```python
from build123d import *

# Parameters (mm, degrees)
TRIANGULAR_BASE_PLATE_DEPTH   = 10
TUBE_SUPPORT_BLOCK_PROFILE_W  = 16
TUBE_SUPPORT_BLOCK_PROFILE_H  = 10
TUBE_SUPPORT_BLOCK_DEPTH      = 55
SUPPORT_WEB_PROFILE_W         = 16
SUPPORT_WEB_PROFILE_H         = 6
SUPPORT_WEB_DEPTH             = 55
TUBE_PROFILE_32_R             = 16
ROUND_TUBE_32_DEPTH           = 55
TUBE_START                    = 30
TUBE_EXTENSION_PROFILE_32_R   = 16
TUBE_EXTENSION_32_DEPTH       = 30
TUBE_BORE_PROFILE_21_R        = 10.5
TUBE_BORE_21_DEPTH            = 85
MOUNTING_HOLES_PROFILE_3X_8_R = 4
MOUNTING_HOLES_3X_8_DEPTH     = 85


with BuildPart() as part:
    # Base Plate Profile → Triangular Base Plate (new body)
    with BuildSketch(Plane.XY):
        with BuildLine():
            Line((-50.21997456, -52.0500159), (-12.71997456, 7.9499841))
            ThreePointArc((-12.71997456, 7.9499841), (0, 15), (12.71997456, 7.9499841))
            Line((12.71997456, 7.9499841), (50.21997456, -52.0500159))
            ThreePointArc((50.21997456, -52.0500159), (50.619637219, -67.271527986), (37.5, -75))
            Line((37.5, -75), (-37.5, -75))
            ThreePointArc((-37.5, -75), (-50.619637219, -67.271527986), (-50.21997456, -52.0500159))
        make_face()
    extrude(amount=TRIANGULAR_BASE_PLATE_DEPTH)

    # Tube Support Block Profile → Tube Support Block (add)
    with BuildSketch(Plane.XZ.offset(75)):
        with Locations((-8, 15)):
            Rectangle(TUBE_SUPPORT_BLOCK_PROFILE_W, TUBE_SUPPORT_BLOCK_PROFILE_H)
        with Locations((8, 15)):
            Rectangle(TUBE_SUPPORT_BLOCK_PROFILE_W, TUBE_SUPPORT_BLOCK_PROFILE_H)
    extrude(amount=-TUBE_SUPPORT_BLOCK_DEPTH)

    # Support Web Profile → Support Web (add)
    with BuildSketch(Plane.XZ.offset(75)):
        with Locations((-8, 23)):
            Rectangle(SUPPORT_WEB_PROFILE_W, SUPPORT_WEB_PROFILE_H)
        with Locations((8, 23)):
            Rectangle(SUPPORT_WEB_PROFILE_W, SUPPORT_WEB_PROFILE_H)
    extrude(amount=-SUPPORT_WEB_DEPTH)

    # Tube Profile Ø32 → Round Tube Ø32 (add)
    with BuildSketch(Plane.XZ.offset(75)):
        with Locations((0, 26)):
            Circle(TUBE_PROFILE_32_R)
    extrude(amount=-ROUND_TUBE_32_DEPTH)

    # Tube Extension Profile Ø32 → Tube Extension Ø32 (add)
    with BuildSketch(Plane.XZ.offset(75).offset(TUBE_START)):
        with Locations(Location((0, 26, 0), (0, 0, 270))):
            Circle(TUBE_EXTENSION_PROFILE_32_R)
    extrude(amount=-TUBE_EXTENSION_32_DEPTH)

    # Tube Bore Profile Ø21 → Tube Bore Ø21 (cut)
    with BuildSketch(Plane.XZ.offset(105)):
        with Locations(Location((0, 26, 0), (0, 0, 270))):
            Circle(TUBE_BORE_PROFILE_21_R)
    extrude(amount=-TUBE_BORE_21_DEPTH, mode=Mode.SUBTRACT)

    # Mounting Holes Profile 3xØ8 → Mounting Holes 3xØ8 (cut)
    with BuildSketch(Plane.XY.offset(10)):
        Circle(MOUNTING_HOLES_PROFILE_3X_8_R)
        with Locations((-37.5, -60)):
            Circle(MOUNTING_HOLES_PROFILE_3X_8_R)
        with Locations((37.5, -60)):
            Circle(MOUNTING_HOLES_PROFILE_3X_8_R)
    extrude(amount=-MOUNTING_HOLES_3X_8_DEPTH, mode=Mode.SUBTRACT)


solid = part.part
```
Work out the finished part from the listing and answer in its coordinate system (mm). A direction names the side the tool comes from. Coordinates: 2 decimals unless noted, no trailing zeros. Loops run counter-clockwise (first coordinate to the right, second up) from the corner with the lowest first, then second, coordinate; pieces in that order, holes last.
1) Flat-ended cylindrical pins translate along their axes: pin 1 (1.5 mm diameter, centred on x = 14, y = -49, fed in from -Z); pin 2 (5 mm diameter, centred on y = -42.5, z = 19.5, fed in from -X); pin 3 (1 mm diameter, centred on y = -80.5, z = 27.5, fed in from +X); pin 4 (1.5 mm diameter, centred on x = -23, y = -39, fed in from +Z). Find the tip coordinate at first contact, or state that the pin passes through.
Results:
pin 1: stops at z = 0
pin 2: stops at x = -16
pin 3: stops at x = 15.97
pin 4: stops at z = 10
2) Section D-D (y = -47.5) is taken. Give the vertices of the cut face in (x, z), plus the area to 3 significant figures.
Results:
outline: (-47.38, 0) - (47.38, 0) - (47.38, 10) - (16, 10) - (16, 26) arc R16 ccw to (-16, 26) - (-16, 10) - (-47.38, 10) - close; hole circle Ø21 at (0, 26)
area: 1,520 mm2
3) Consider probe 1 along Z at (x, y) = (0.5, -99); probe 2 along X at (y, z) = (-79, 26); probe 3 along Z at (x, y) = (-25, -43). Determine where each line is inside the solid, lowest interval first.
Results:
probe 1: z = 10.01 to 15.51, 36.49 to 41.99
probe 2: x = -16 to -10.5, 10.5 to 16
probe 3: z = 0 to 10
4) Section B-B (x = 0) is taken. Give the vertices of the cut face in (y, z), plus the area to 4 significant figures.
Results:
outline: (-105, 10) - (-75, 10) - (-75, 0) - (-4, 0) - (-4, 10) - (-20, 10) - (-20, 15.5) - (-105, 15.5) - close; (-105, 36.5) - (-20, 36.5) - (-20, 42) - (-105, 42) - close; (4, 0) - (15, 0) - (15, 10) - (4, 10) - close
area: 1,755 mm2
5) Section C-C (z = 17.5) is taken. Give the vertices of the cut face in (x, y), plus the area to 3 significant figures.
Results:
outline: (-16, -75) - (-13.56, -75) - (-13.56, -105) - (-6.16, -105) - (-6.16, -20) - (-16, -20) - close; (6.16, -105) - (13.56, -105) - (13.56, -75) - (16, -75) - (16, -20) - (6.16, -20) - close
area: 1,530 mm2
6) For faces 4 (the flat face through (3.3, -20, 15.6)), 5 (the flat face through (-16, -48, 18)), 6 (the cylindrical face through (0, 15, 5)), 7 (the flat face through (16, -48, 18)), 8 (the cylindrical face through (0.703, -72.539, 41.985)), determine the directions among +Z, -Z, +X, -X, +Y, -Y from which every point of the face is accessible in a straight line to the end or side of a thin tool.
Results:
face 4: +Z, +X, -X, +Y
face 5: +Z, -X, +Y, -Y
face 6: +Z, -Z, +Y
face 7: +Z, +X, +Y, -Y
face 8: -Y
7) For a pull along Y with two mould halves and no side action, classify faces 1 (the flat face through (-3.3, -105, 15.6)), 2 (the flat face through (1, -39, 0)), 3 (the cylindrical face through (-38.367, -63.905, 5.07)) as +Y half, -Y half, draft (parallel to the pull), parting line (faces both ways), or undercut.
Results:
face 1: -Y half
face 2: draft
face 3: undercut
8) Section A-A (y = -60) is taken. Give the vertices of the cut face in (x, z).
Results:
outline: (-52.5, 0) - (-41.5, 0) - (-41.5, 10) - (-52.5, 10) - close; (-33.5, 0) - (33.5, 0) - (33.5, 10) - (16, 10) - (16, 26) arc R16 ccw to (-16, 26) - (-16, 10) - (-33.5, 10) - close; (41.5, 0) - (52.5, 0) - (52.5, 10) - (41.5, 10) - close; hole circle Ø21 at (0, 26)
